Can you work these out from the model? Positions are in its coordinate system, mm. Face numbers are marked on the shaded views. Coordinates: 2 decimals unless noted, no trailing zeros. Write each loop counter-clockwise with the first axis right and the second up, starting at its lowest first coordinate (ties: lowest second). Pieces come first, ordered by that corner, then holes. Notation, with made-up numbers: (76.5, 73.5) - (123.5, 73.5) arc R24 cw to (123.5, 109.5) - close; hole circle Ø10 at (34, 45). An arc over 180 degrees is marked (long way). One line per question, with ' | ' between items. Start each with the question number.
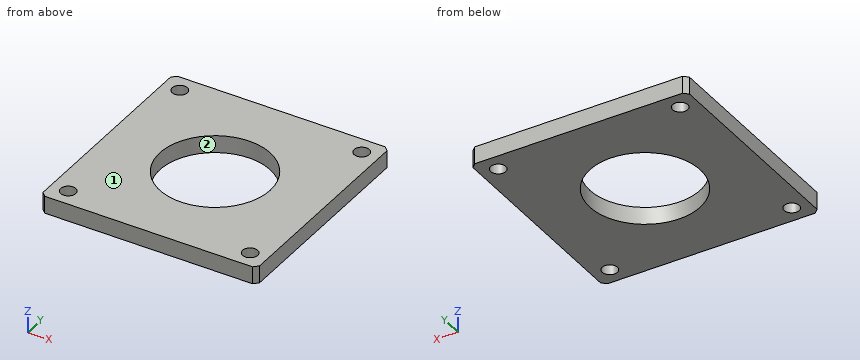
from build123d import *

# Parameters (mm, degrees)
SKETCH_1_W               = 100
SKETCH_1_H               = 100
EXTRUDE_1_DEPTH          = 8
CUT_EXTRUDE_1_REACH      = 73.162
SKETCH_2_R               = 25.5
CUT_EXTRUDE_2_REACH      = 73.162
SKETCH_3_R               = 3.5
PATTERN_CIRCULAR_1_COUNT = 4
CHAMFER_1_SIZE           = 2


with BuildPart() as part:
    # 草图1 → 凸台-拉伸1 (new body)
    with BuildSketch(Plane.XY):
        Rectangle(SKETCH_1_W, SKETCH_1_H)
    extrude(amount=EXTRUDE_1_DEPTH)

    # 草图2 → 切除-拉伸1 (cut, up to next)
    with BuildSketch(Plane.XY.offset(8), mode=Mode.PRIVATE) as cut_extrude_1_sk1:
        Circle(SKETCH_2_R)
    cut_extrude_1_tool1 = extrude(cut_extrude_1_sk1.sketch, amount=-CUT_EXTRUDE_1_REACH, mode=Mode.PRIVATE) & part.part
    add(cut_extrude_1_tool1.solids().sort_by_distance((0, 0, 8))[0], mode=Mode.SUBTRACT)

    # 草图3 → 切除-拉伸2 (cut, up to next)
    with BuildSketch(Plane.XY.offset(8), mode=Mode.PRIVATE) as cut_extrude_2_sk1:
        with Locations((-42, 42)):
            Circle(SKETCH_3_R)
    cut_extrude_2_tool1 = extrude(cut_extrude_2_sk1.sketch, amount=-CUT_EXTRUDE_2_REACH, mode=Mode.PRIVATE) & part.part
    cut_extrude_2 = cut_extrude_2_tool1.solids().sort_by_distance((-42, 42, 8))[0]
    add(cut_extrude_2, mode=Mode.SUBTRACT)

    # 阵列(圆周)1: 切除-拉伸2 ×4 about axis
    pattern_circular_1_axis = Axis((0, 0, 0), (0, 0, 1))
    for i in range(1, PATTERN_CIRCULAR_1_COUNT):
        add(cut_extrude_2.rotate(pattern_circular_1_axis, i * 360 / PATTERN_CIRCULAR_1_COUNT), mode=Mode.SUBTRACT)

    # 倒角1
    chamfer_1_edges = [part.edges().sort_by_distance(p)[0] for p in [
        (50, -50, 4),
        (-50, -50, 4),
        (-50, 50, 4),
        (50, 50, 4),
    ]]
    chamfer(chamfer_1_edges, length=CHAMFER_1_SIZE)


solid = part.part
(1) If we section it at C-C on y = -42: List the corners of the cut face in (x, z) for me.
(2) If I drill on probe 1 along Y at (x, z) = (-42, 2.25); probe 2 along Y at (x, z) = (-39, 7.25), over which ranges is the centre line in solid material (lowest first)?
(3) If we mould it in two halves opening along X, with no side actions, what happens to the marked faces 1 and 2? For each: +X half, -X half, draft (parallel to the pull), parting line (faces both ways), or undercut.
(4) I'm going to push a flat-ended pin straight in: pin 1 (4 mm diameter, centred on x = -42, y = -42, fed in from -Z). Where does the tip first touch, or does it pass through?
(5) If we section it at B-B on z = 6.75: List the corners of the cut face in (x, y) for me.
(6) If we section it at A-A on x = -12: List the corners of the cut face in (y, z) for me.
Values:
1) outline: (-50, 0) - (-45.5, 0) - (-45.5, 8) - (-50, 8) - close; (-38.5, 0) - (38.5, 0) - (38.5, 8) - (-38.5, 8) - close; (45.5, 0) - (50, 0) - (50, 8) - (45.5, 8) - close
2) probe 1: -50 to -45.5, -38.5 to 38.5, 45.5 to 50 | probe 2: -50 to -43.8, -40.2 to 40.2, 43.8 to 50
3) face 1: draft | face 2: undercut
4) pin 1: through
5) outline: (-50, -48) - (-48, -50) - (48, -50) - (50, -48) - (50, 48) - (48, 50) - (-48, 50) - (-50, 48) - close; hole circle Ø7 at (-42, -42); hole circle Ø7 at (-42, 42); hole circle Ø51 at (0, 0); hole circle Ø7 at (42, -42); hole circle Ø7 at (42, 42)
6) outline: (-50, 0) - (-22.5, 0) - (-22.5, 8) - (-50, 8) - close; (22.5, 0) - (50, 0) - (50, 8) - (22.5, 8) - close
